```python
from build123d import *

# Parameters (mm, degrees)
HUB_PROFILE_SKETCH_W                   = 7
HUB_PROFILE_SKETCH_H                   = 3
PLATE_OUTLINE_SKETCH_65X50_OUTSIDE_W   = 85.506
PLATE_OUTLINE_SKETCH_65X50_OUTSIDE_H   = 85.506
PLATE_OUTLINE_SKETCH_65X50_OUTSIDE_W_2 = 65
PLATE_OUTLINE_SKETCH_65X50_OUTSIDE_H_2 = 50
HUB_TRIM_CUT_65X50_DEPTH               = 10
BASE_PLATE_SKETCH_65X50_W              = 65
BASE_PLATE_SKETCH_65X50_H              = 50
BASE_PLATE_65X50X3_DEPTH               = 3
PLATE_CORNER_FILLETS_R6_R              = 6
MOUNTING_HOLES_SKETCH_R                = 2.5
MOUNTING_HOLES_4X_DEPTH                = 3
MOUNTING_HOLE_CHAMFERS_1_5X45_SIZE     = 1.5
CENTER_BORE_SKETCH_R                   = 9.879541092
CENTER_BORE_CUT_DEPTH                  = 23
HUB_GROOVE_SKETCH_45_R                 = 22.5
HUB_GROOVE_45_DEPTH                    = 3
SKETCH3_2_W                            = 65
SKETCH3_2_H                            = 50
PLATE_STEP_65X50X3_DEPTH               = 3


with BuildPart() as part:
    # Hub Profile Sketch → Hub Revolve (revolve)
    with BuildSketch(Plane.XY, mode=Mode.PRIVATE) as hub_revolve_sk:
        with Locations((3.5, 9.089822415)):
            Rectangle(HUB_PROFILE_SKETCH_W, HUB_PROFILE_SKETCH_H)
        with BuildLine():
            Line((9.879541092, 10.589822415), (7, 10.589822415))
            Line((7, 10.589822415), (7, 7.589822415))
            Line((7, 7.589822415), (9.879541092, 7.589822415))
            ThreePointArc((9.879541092, 7.589822415), (11.931661952, 7.22797814), (13.73626675, 6.186089074))
            Line((13.73626675, 6.186089074), (18.599204249, 2.105600012))
            ThreePointArc((18.599204249, 2.105600012), (21.306111446, 0.542766413), (24.384292736, 0))
            Line((24.384292736, 0), (32.5, 0))
            Line((32.5, 0), (32.5, 3))
            Line((32.5, 3), (24.384292736, 3))
            ThreePointArc((24.384292736, 3), (22.332171876, 3.361844275), (20.527567078, 4.403733341))
            Line((20.527567078, 4.403733341), (15.664629579, 8.484222403))
            ThreePointArc((15.664629579, 8.484222403), (12.957722382, 10.047056002), (9.879541092, 10.589822415))
        make_face()
    revolve(hub_revolve_sk.sketch.rotate(Axis((0, 0, 0), (0, 1, 0)), 90), axis=Axis((0, 0, 0), (0, 1, 0)))

    # Plate Outline Sketch 65x50 outside → Hub Trim Cut 65x50 (cut)
    with BuildSketch(Plane(origin=(0, 3, 0), x_dir=(1, 0, 0), z_dir=(0, 1, 0))):
        Rectangle(PLATE_OUTLINE_SKETCH_65X50_OUTSIDE_W, PLATE_OUTLINE_SKETCH_65X50_OUTSIDE_H)
        Rectangle(PLATE_OUTLINE_SKETCH_65X50_OUTSIDE_W_2, PLATE_OUTLINE_SKETCH_65X50_OUTSIDE_H_2, mode=Mode.SUBTRACT)
    extrude(amount=-HUB_TRIM_CUT_65X50_DEPTH, mode=Mode.SUBTRACT)

    # Base Plate Sketch 65x50 → Base Plate 65x50x3 (add)
    with BuildSketch(Plane(origin=(0, 3, 0), x_dir=(1, 0, 0), z_dir=(0, 1, 0))):
        Rectangle(BASE_PLATE_SKETCH_65X50_W, BASE_PLATE_SKETCH_65X50_H)
    extrude(amount=-BASE_PLATE_65X50X3_DEPTH)

    # Plate Corner Fillets R6
    plate_corner_fillets_r6_edges = [part.edges().sort_by_distance(p)[0] for p in [
        (32.5, 1.5, -25),
        (32.5, 1.5, 25),
        (-32.5, 1.5, 25),
        (-32.5, 1.5, -25),
    ]]
    fillet(plate_corner_fillets_r6_edges, radius=PLATE_CORNER_FILLETS_R6_R)

    # Mounting Holes Sketch → Mounting Holes 4x (cut)
    with BuildSketch(Plane(origin=(0, 3, 0), x_dir=(1, 0, 0), z_dir=(0, 1, 0))):
        with Locations(Location((-26.5, 19, 0), (0, 0, 270))):
            Circle(MOUNTING_HOLES_SKETCH_R)
        with Locations(Location((26.5, 19, 0), (0, 0, 270))):
            Circle(MOUNTING_HOLES_SKETCH_R)
        with Locations(Location((26.5, -19, 0), (0, 0, 270))):
            Circle(MOUNTING_HOLES_SKETCH_R)
        with Locations(Location((-26.5, -19, 0), (0, 0, 270))):
            Circle(MOUNTING_HOLES_SKETCH_R)
    extrude(amount=-MOUNTING_HOLES_4X_DEPTH, mode=Mode.SUBTRACT)

    # Mounting Hole Chamfers 1.5x45
    mounting_hole_chamfers_1_5x45_edges = [part.edges().sort_by_distance(p)[0] for p in [
        (-26.5, 3, 16.5),
        (26.5, 3, 16.5),
        (26.5, 3, -21.5),
        (-26.5, 3, -21.5),
    ]]
    chamfer(mounting_hole_chamfers_1_5x45_edges, length=MOUNTING_HOLE_CHAMFERS_1_5X45_SIZE)

    # Center Bore Sketch → Center Bore Cut (cut)
    with BuildSketch(Plane(origin=(0, 10.589822415, 0), x_dir=(1, 0, 0), z_dir=(0, 1, 0))):
        with Locations(Location((0, 0, 0), (0, 0, 90))):
            Circle(CENTER_BORE_SKETCH_R)
    extrude(amount=-CENTER_BORE_CUT_DEPTH, mode=Mode.SUBTRACT)

    # Hub Groove Sketch _45 → Hub Groove _45 (cut)
    with BuildSketch(Plane.XZ):
        with Locations(Location((0, 0, 0), (0, 0, 270))):
            Circle(HUB_GROOVE_SKETCH_45_R)
    extrude(amount=-HUB_GROOVE_45_DEPTH, mode=Mode.SUBTRACT)

    # Sketch3_2 → Plate Step 65x50x3 (add)
    with BuildSketch(Plane(origin=(0, 3, 0), x_dir=(1, 0, 0), z_dir=(0, 1, 0))):
        Rectangle(SKETCH3_2_W, SKETCH3_2_H)
    extrude(amount=-PLATE_STEP_65X50X3_DEPTH)


solid = part.part
```
Model file for the job. Use its own axes, mm. Round coordinates to 2 decimals unless told otherwise and drop trailing zeros. Write each loop counter-clockwise with the first axis right and the second up, starting at its lowest first coordinate (ties: lowest second). Pieces come first, ordered by that corner, then holes. Notation, with made-up numbers: M 79,85.5 L 113,85.5 A21 cw 113,119.5 Z; hole C 68,-39 d4. An arc over 180 degrees is marked long. Put each result on its own line as item: value.
Item 1: Cut at B-B (z = 0). List the corners of the cut face in (x, y), and give its area (3 significant figures).
Responses:
outline: M -32.5,0 L 32.5,0 L 32.5,3 L 24.38,3 A6 cw 20.53,4.4 L 15.66,8.48 A9 ccw 9.88,10.59 L 9.88,7.59 A6 cw 13.74,6.19 L 17.53,3 L -17.53,3 L -13.74,6.19 A6 cw -9.88,7.59 L -9.88,10.59 A9 ccw -15.66,8.48 L -20.53,4.4 A6 cw -24.38,3 L -32.5,3 Z
area: 268 mm²
Item 2: Cut at A-A (x = 0). List the corners of the cut face in (y, z), and give its area (3 significant figures).
Responses:
outline: M 0,-25 L 3,-25 L 3,-24.38 A6 cw 4.4,-20.53 L 8.48,-15.66 A9 ccw 10.59,-9.88 L 7.59,-9.88 A6 cw 6.19,-13.74 L 3,-17.53 L 3,17.53 L 6.19,13.74 A6 cw 7.59,9.88 L 10.59,9.88 A9 ccw 8.48,15.66 L 4.4,20.53 A6 cw 3,24.38 L 3,25 L 0,25 Z
area: 223 mm²
Item 3: Probe L1, parallel to Z at x = -4.5, y = 8.5; L2, parallel to Y at x = -25, z = -21; L3, parallel to X at y = 9.5, z = 0. List the from-to ranges inside material, lowest first. Write a range as from..to.
Responses:
L1: -14.98..-8.8, 8.8..14.98
L2: 0..3
L3: -14.17..-9.88, 9.88..14.17
Item 4: Mould opens along Y. For faces 1 (the flat face through (0, 3, 0)), 2 (the flat face through (-22, 3, -11)), 3 (the conical face through (12.397, 5.987, -6.448)), 4 (the cylindrical face through (8.765, 9.111, -4.559)) say: +Y half, -Y half, draft (parallel to the pull), parting line (faces both ways), or undercut.
Responses:
face 1: undercut
face 2: +Y half
face 3: undercut
face 4: draft
Item 5: Flat gauge pins, fed straight in: P1, Ø2, axis at x = 7, y = 5, coming from the +Z side; P2, Ø16, axis at x = 0, z = 0, coming from the +Y side; P3, Ø6, axis at x = -22.5, z = 1, coming from the +Y side. Where does each tip first touch, or does it go through?
Responses:
P1: z = 19.91
P2: y = 3
P3: y = 5.25
